Build history of the part. All positions in model axes, mm. Face numbers are marked on the shaded views. A direction names the side the tool comes from. Coordinates: 2 decimals unless noted, no trailing zeros. Order: outer loops, then holes, each group sorted by start corner. A loop starts at its lowest first (then second) coordinate and runs counter-clockwise, first axis right, second up. Notation, with made-up numbers: (-22.5, 4.5) - (30.5, 4.5) arc R17 cw to (30.5, 9.5) - close; hole circle Ø8 at (-36, 12.25). An arc over 180 degrees is marked (long way). Answer as CSV lines item,"result". Start each with the question number.
from build123d import *

# Parameters (mm, degrees)
LEVER_PLATE_DEPTH           = 16
FRONT_HUB_SKETCH_40_R       = 40
FRONT_PIVOT_HUB_40_DEPTH    = 8
REAR_START                  = 16
REAR_HUB_SKETCH_40_R        = 40
REAR_PIVOT_HUB_40_DEPTH     = 16
SMALL_HOLE_SKETCH_8_R       = 8
SMALL_HOLE_8_DEPTH          = 16
SMALL_HOLE_CHAMFER_2MM_SIZE = 2
EYE_PAD_74X74_DEPTH         = 15
EYE_BLOCK_DEPTH             = 60
EYE_BORE_SKETCH_25_R        = 25
EYE_BORE_25_DEPTH           = 60
PIVOT_BORE_SKETCH_20_R      = 20
PIVOT_BORE_20_DEPTH         = 40


with BuildPart() as part:
    # Lever Plate Profile → Lever Plate (new body)
    with BuildSketch(Plane.XY):
        with BuildLine():
            Line((143.896503384, 61.42345762), (6.758164717, 99.929217055))
            ThreePointArc((6.758164717, 99.929217055), (-13.046071322, 97.186040961), (-24.506399585, 80.803316636))
            Line((-24.506399585, 80.803316636), (-39.210239337, 7.909306617))
            ThreePointArc((-39.210239337, 7.909306617), (-30.954581767, -25.334045623), (0, -40))
            Line((0, -40), (129.839520773, -40.640513855))
            ThreePointArc((129.839520773, -40.640513855), (181.3532399, 4.26464706), (143.896503384, 61.42345762))
        make_face()
    extrude(amount=LEVER_PLATE_DEPTH)

    # Front Hub Sketch Ø40 → Front Pivot Hub Ø40 (add)
    with BuildSketch(Plane.XY.offset(16)):
        with Locations(Location((0, 0, 0), (0, 0, 168.595597299))):
            Circle(FRONT_HUB_SKETCH_40_R)
    extrude(amount=FRONT_PIVOT_HUB_40_DEPTH)

    # Rear Hub Sketch Ø40 → Rear Pivot Hub Ø40 (add)
    with BuildSketch(Plane(origin=(0, 0, 0), x_dir=(-1, 0, 0), z_dir=(0, 0, -1)).offset(REAR_START)):
        Circle(REAR_HUB_SKETCH_40_R)
    extrude(amount=-REAR_PIVOT_HUB_40_DEPTH)

    # Small Hole Sketch Ø8 → Small Hole Ø8 (cut)
    with BuildSketch(Plane.XY.offset(16)):
        with Locations((0, 75.86)):
            Circle(SMALL_HOLE_SKETCH_8_R)
    extrude(amount=-SMALL_HOLE_8_DEPTH, mode=Mode.SUBTRACT)

    # Small Hole Chamfer 2mm
    small_hole_chamfer_2mm_edges = [part.edges().sort_by_distance(p)[0] for p in [
        (-8, 75.86, 16),
    ]]
    chamfer(small_hole_chamfer_2mm_edges, length=SMALL_HOLE_CHAMFER_2MM_SIZE)

    # Eye Pad Sketch 74x74 → Eye Pad 74x74 (add)
    with BuildSketch(Plane.XY.offset(16)):
        Polygon((92.980316943, 8.134723664), (129.839520773, 11.359486145), (126.614758291, 48.218689975), (89.755554462, 44.993927493), align=None)
        Polygon((126.614758291, 48.218689975), (129.839520773, 11.359486145), (129.839520773, 48.500820134), align=None)
        with BuildLine():
            Line((129.839520773, 48.500820134), (129.839520773, 11.359486145))
            Line((129.839520773, 11.359486145), (92.980316943, 8.134723664))
            Line((92.980316943, 8.134723664), (96.205079425, -28.724480166))
            Line((96.205079425, -28.724480166), (169.462898271, -22.315251502))
            ThreePointArc((169.462898271, -22.315251502), (169.673831815, -22.065469558), (169.883190784, -21.81436639))
            Line((169.883190784, -21.81436639), (163.51425842, 50.982863644))
            ThreePointArc((163.51425842, 50.982863644), (163.264476476, 51.193797187), (163.013373308, 51.403156157))
            Line((163.013373308, 51.403156157), (129.839520773, 48.500820134))
        make_face()
    extrude(amount=EYE_PAD_74X74_DEPTH)

    # Eye Block Sketch → Eye Block (add)
    with BuildSketch(Plane.XY.offset(31)):
        Polygon((89.755554462, 44.993927493), (163.51425842, 50.982863644), (169.883190784, -21.81436639), (96.205079425, -28.724480166), align=None)
    extrude(amount=-EYE_BLOCK_DEPTH)

    # Eye Bore Sketch Ø25 → Eye Bore Ø25 (cut)
    with BuildSketch(Plane.XY.offset(31)):
        with Locations((129.609226366, 11.339337995)):
            Circle(EYE_BORE_SKETCH_25_R)
    extrude(amount=-EYE_BORE_25_DEPTH, mode=Mode.SUBTRACT)

    # Pivot Bore Sketch Ø20 → Pivot Bore Ø20 (cut)
    with BuildSketch(Plane.XY.offset(24)):
        Circle(PIVOT_BORE_SKETCH_20_R)
    extrude(amount=-PIVOT_BORE_20_DEPTH, mode=Mode.SUBTRACT)


solid = part.part
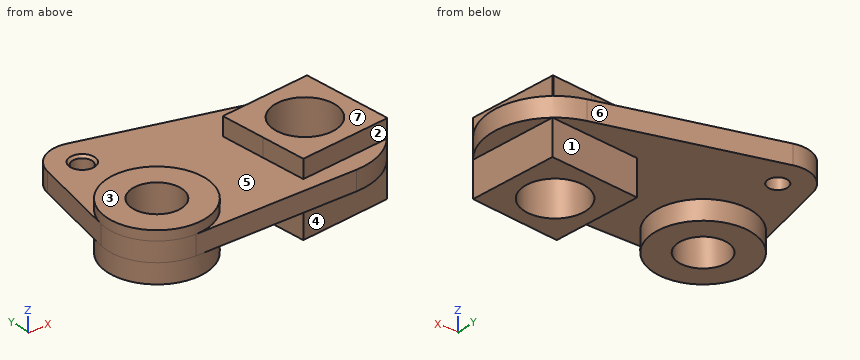
(1) Band-saw the part on A-A on z = 19. List the corners of the cut face in (x, y).
(2) Which spindle directions (+Z, -Z, +X, -X, +Y, -Y) get a long thin tool onto all of the face, cutting with end or side? Do the marked faces 1, 2, 3 and 4. Say none if no direction does.
(3) Drop flat-ended pins along their axis: pin 1 Ø9 at (x, y) = (175.5, 20) entering from +Z; pin 2 Ø1 at (x, y) = (17, 35) entering from +Z; pin 3 Ø4 at (x, z) = (153.5, -20.5) entering from +Y. Give the stop position or say it passes through.
(4) Pull direction X, two halves, no side cores. Call the marked faces 5, 6 and 7: +X half, -X half, draft (parallel to the pull), parting line (faces both ways), or undercut.
(5) Band-saw the part on B-B on x = 134.5. List the corners of the cut face in (y, z).
(6) Band-saw the part on D-D on y = 32.5. List the corners of the cut face in (x, z).
(7) Band-saw the part on C-C on y = 0. List the corners of the cut face in (x, z), plus the area to 3 significant figures.
(8) Probe L1, parallel to X at y = 25.5, z = 22; L2, parallel to X at y = -9.5, z = 20; L3, parallel to Y at x = 0, z = 16.5. List the from-to ranges inside material, lowest first. Write a range as [from, to].
Filled in:
1,outline,"circle Ø80 at (0, 0); (89.76, 44.99) - (96.21, -28.72) - (169.46, -22.32) arc R52 ccw to (169.88, -21.81) - (163.51, 50.98) arc R52 ccw to (163.01, 51.4) - close; hole circle Ø40 at (0, 0); hole circle Ø50 at (129.61, 11.34)"
2,face 1,"-Z, -X, +Y"
2,face 2,"+Z, +X, -Y"
2,face 3,"+Z, -X, +Y, -Y"
2,face 4,"-Z, +X, -Y"
3,pin 1,"stops at z = 16"
3,pin 2,"stops at z = 24"
3,pin 3,"stops at y = 50.33"
4,face 5,"undercut"
4,face 6,"+X half"
4,face 7,"draft"
5,outline,"(-40.43, 0) - (-25.13, 0) - (-25.13, -29) - (-13.18, -29) - (-13.18, 31) - (-25.37, 31) - (-25.37, 16) - (-40.43, 16) - close; (35.86, -29) - (48.63, -29) - (48.63, 0) - (64.06, 0) - (64.06, 16) - (48.91, 16) - (48.91, 31) - (35.86, 31) - close"
6,outline,"(-34.25, 0) - (-23.32, 0) - (-23.32, -16) - (23.32, -16) - (23.32, 0) - (90.85, 0) - (90.85, -29) - (116.3, -29) - (116.3, 31) - (90.85, 31) - (90.85, 16) - (23.32, 16) - (23.32, 24) - (-23.32, 24) - (-23.32, 16) - (-34.25, 16) - close; (142.92, -29) - (165.13, -29) - (165.13, 0) - (177.35, 0) - (177.35, 16) - (165.13, 16) - (165.13, 31) - (142.92, 31) - close"
7,outline,"(-40, -16) - (-20, -16) - (-20, 24) - (-40, 24) - close; (20, -16) - (40, -16) - (40, 0) - (93.69, 0) - (93.69, -29) - (107.33, -29) - (107.33, 31) - (93.69, 31) - (93.69, 16) - (40, 16) - (40, 24) - (20, 24) - close; (151.89, -29) - (167.97, -29) - (167.97, 0) - (180.58, 0) - (180.58, 16) - (167.97, 16) - (167.97, 31) - (151.89, 31) - close"
7,area,"4,440 mm^2"
8,L1,"x = [-30.82, 30.82], [91.46, 109.01], [150.21, 165.74]"
8,L2,"x = [-38.86, -17.6], [17.6, 38.86], [94.52, 115.8], [143.42, 168.81]"
8,L3,"y = [-40, -20], [20, 40]"
